Can you work these out from the model? Positions are in its coordinate system, mm. A direction names the side the tool comes from. Coordinates: 2 decimals unless noted, no trailing zeros. Order: outer loops, then holes, each group sorted by start corner. A loop starts at its lowest first (then second) coordinate and runs counter-clockwise, first axis right, second up. Notation, with made-up numbers: (26.25, -16.75) -> (32.25, -16.75) arc R11 ccw to (32.25, -3.75) -> close; hole circle Ø11 at (14.25, 87.25). An arc over 180 degrees is marked (long way). Answer as a JSON object with one key per item and string values. Group by question number.
(1) Which directions (+Z, -Z, +X, -X, +Y, -Y) give clear straight access to the entire face, cutting with the end or side of a thin tool? Please do faces 1 (the flat face through (423, -4, -4)), 2 (the flat face through (-202, 0, 0)), 3 (the cylindrical face through (368.689, -19.334, -2.539)), 4 (the flat face through (-40, 0, 13.55)), 5 (the cylindrical face through (-125.95, 17.847, -2.343)).
(2) I want a section at A-A, the plane x = -96. List the corners of the cut face in (y, z) for me.
(3) I need wall thicknesses on line 1 (X direction, y = 0, z = 13); line 2 (Y direction, x = 411.25, z = 0); line 3 (Z direction, x = 407.5, y = 0). Which ranges of each line are inside material? Lowest first, please.
(4) I want a section at B-B, the plane x = 21. List the corners of the cut face in (y, z) for me.
(5) If we mould it in two halves opening along Y, with no side actions, what happens to faces 6 (the flat face through (402, 0, 11.77)), 7 (the cylindrical face through (-191.864, 1.532, 7.86)), 8 (the flat face through (-27, 4.4, -19.2)), 9 (the cylindrical face through (167.62, 22.804, 2.994))? For each: pulls with the +Y half, pulls with the -Y half, needs draft (parallel to the pull), parting line crosses it, or undercut.
(6) For pin 1 (2 mm diameter, centred on x = 56.5, z = -16, fed in from -Y); pin 2 (1.5 mm diameter, centred on x = 399, z = 13.5, fed in from +Y); pin 3 (6 mm diameter, centred on x = -42.5, y = -2.5, fed in from +Z); pin 4 (12 mm diameter, centred on y = -2.5, z = 3, fed in from +X), each with a flat end and sliding along its axis, tell me the tip position at first contact or that it passes through.
from build123d import *

# Parameters (mm, degrees)
SKETCH_1_R               = 23
EXTRUDE_1_DEPTH          = 340
SKETCH_2_R               = 20
EXTRUDE_2_DEPTH          = 27
SKETCH_3_R               = 19.5
EXTRUDE_3_DEPTH          = 25
EXTRUDE_START            = 15
SKETCH_4_R               = 20
EXTRUDE_4_DEPTH          = 15
EXTRUDE_START_2          = 27
SKETCH_5_R               = 19.5
EXTRUDE_5_DEPTH          = 27
SKETCH_6_R               = 17.5
EXTRUDE_6_DEPTH          = 41
CUT_EXTRUDE_1_DEPTH      = 5.73
SKETCH_8_R               = 18
EXTRUDE_7_DEPTH          = 150
HOLE_WIZARD_M12_2_D      = 10.2
HOLE_WIZARD_M12_2_DEPTH  = 20
HOLE_WIZARD_M12_2_TIP    = 3.064389157
HOLE_WIZARD_M10_1_D      = 8.5
HOLE_WIZARD_M10_1_DEPTH  = 20
HOLE_WIZARD_M10_1_TIP    = 2.553657631
CUT_EXTRUDE_2_DEPTH      = 5
CUT_EXTRUDE_2_DEPTH_BACK = 3.95


with BuildPart() as part:
    # 草图1 → 凸台-拉伸1 (new body)
    with BuildSketch(Plane(origin=(0, 0, 0), x_dir=(0, 0, -1), z_dir=(1, 0, 0))):
        Circle(SKETCH_1_R)
    extrude(amount=EXTRUDE_1_DEPTH)

    # 草图2 → 凸台-拉伸2 (add)
    with BuildSketch(Plane.ZY):
        with Locations(Location((0, 0, 0), (0, 0, 180))):
            Circle(SKETCH_2_R)
    extrude(amount=EXTRUDE_2_DEPTH)

    # 草图3 → 凸台-拉伸3 (add)
    with BuildSketch(Plane.ZY.offset(27)):
        Circle(SKETCH_3_R)
    extrude(amount=EXTRUDE_3_DEPTH)

    # 草图4 → 凸台-拉伸4 (add)
    with BuildSketch(Plane(origin=(340, 0, 0), x_dir=(0, 0, -1), z_dir=(1, 0, 0)).offset(EXTRUDE_START)):
        Circle(SKETCH_4_R)
    extrude(amount=-EXTRUDE_4_DEPTH)

    # 草图5 → 凸台-拉伸5 (add)
    with BuildSketch(Plane(origin=(355, 0, 0), x_dir=(0, 0, -1), z_dir=(1, 0, 0)).offset(EXTRUDE_START_2)):
        with Locations(Location((0, 0, 0), (0, 0, 180))):
            Circle(SKETCH_5_R)
    extrude(amount=-EXTRUDE_5_DEPTH)

    # 草图6 → 凸台-拉伸6 (add)
    with BuildSketch(Plane(origin=(382, 0, 0), x_dir=(0, 0, -1), z_dir=(1, 0, 0))):
        Circle(SKETCH_6_R)
    extrude(amount=EXTRUDE_6_DEPTH)

    # 草图7 → 切除-拉伸1 (cut)
    with BuildSketch(Plane.XY.offset(17.5)):
        with BuildLine():
            Line((389, 5), (415, 5))
            ThreePointArc((415, 5), (420, 0), (415, -5))
            Line((415, -5), (389, -5))
            ThreePointArc((389, -5), (384, 0), (389, 5))
        make_face()
    extrude(amount=-CUT_EXTRUDE_1_DEPTH, mode=Mode.SUBTRACT)

    # 草图8 → 凸台-拉伸7 (add)
    with BuildSketch(Plane.ZY.offset(52)):
        Circle(SKETCH_8_R)
    extrude(amount=EXTRUDE_7_DEPTH)

    # M12 螺纹孔2
    with Locations(Plane.XY.offset(18)):
        with Locations((-187, 0)):
            Hole(HOLE_WIZARD_M12_2_D / 2, depth=HOLE_WIZARD_M12_2_DEPTH)
            with Locations((0, 0, -(HOLE_WIZARD_M12_2_DEPTH + HOLE_WIZARD_M12_2_TIP / 2))):  # 118° drill point
                Cone(0, HOLE_WIZARD_M12_2_D / 2, HOLE_WIZARD_M12_2_TIP, mode=Mode.SUBTRACT)

    # M10 螺纹孔1
    with Locations(Plane(origin=(423, 0, 0), x_dir=(0, 0, -1), z_dir=(1, 0, 0))):
        with Locations((0, 0)):
            Hole(HOLE_WIZARD_M10_1_D / 2, depth=HOLE_WIZARD_M10_1_DEPTH)
            with Locations((0, 0, -(HOLE_WIZARD_M10_1_DEPTH + HOLE_WIZARD_M10_1_TIP / 2))):  # 118° drill point
                Cone(0, HOLE_WIZARD_M10_1_D / 2, HOLE_WIZARD_M10_1_TIP, mode=Mode.SUBTRACT)

    # 草图18 → 切除-拉伸2 (cut, two sides: drawn at the far end of the back side and taken through both)
    with BuildSketch(Plane.XY.offset(17.5).offset(-CUT_EXTRUDE_2_DEPTH_BACK)):
        with BuildLine():
            Line((-36, -6), (-44, -6))
            ThreePointArc((-44, -6), (-50, 0), (-44, 6))
            Line((-44, 6), (-36, 6))
            ThreePointArc((-36, 6), (-30, 0), (-36, -6))
        make_face()
    extrude(amount=CUT_EXTRUDE_2_DEPTH + CUT_EXTRUDE_2_DEPTH_BACK, mode=Mode.SUBTRACT)


solid = part.part
Computed values:
{
 "1": {"face 1": "+Z, -Z, +X, +Y, -Y", "face 2": "+Z, -Z, -X, +Y, -Y", "face 3": "+X", "face 4": "+Z", "face 5": "-X"},
 "2": {"outline": "circle Ø36 at (0, 0)"},
 "3": {"line 1": "x = -202 to -192.1, -181.9 to 384, 420 to 423", "line 2": "y = -17.5 to -4.25, 4.25 to 17.5", "line 3": "z = -17.5 to -4.25, 4.25 to 11.77"},
 "4": {"outline": "circle Ø46 at (0, 0)"},
 "5": {"face 6": "undercut", "face 7": "undercut", "face 8": "needs draft", "face 9": "parting line crosses it"},
 "6": {"pin 1": "stops at y = -17.44", "pin 2": "stops at y = 11.99", "pin 3": "stops at z = 13.55", "pin 4": "stops at x = 423"}
}
